Can you work these out from the model? Positions are in its coordinate system, mm. Face numbers are marked on the shaded views. A direction names the side the tool comes from. Round coordinates to 2 decimals unless told otherwise and drop trailing zeros. Order: outer loops, then holes, each group sorted by start corner. A loop starts at its lowest first (then second) coordinate and runs counter-clockwise, first axis right, second up. Notation, with made-up numbers: (36.25, 35) -> (67.25, 35) arc R16 cw to (67.25, 44) -> close; hole circle Ø2 at (-2.5, -31.75). An arc over 180 degrees is marked (long way). One line per item, written item: value.
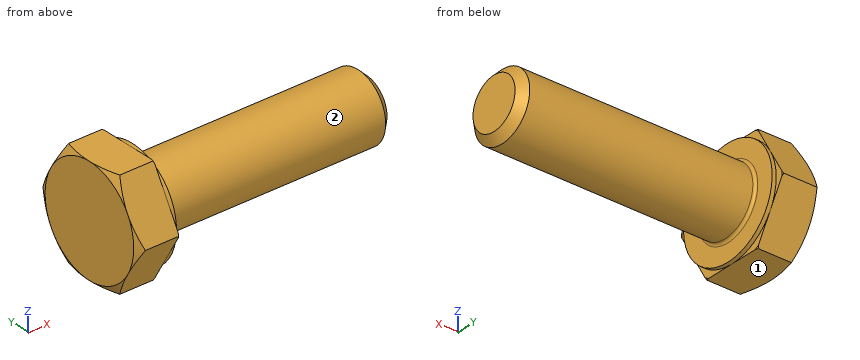
```python
from build123d import *

# Parameters (mm, degrees)
EXTRUDE_368_DEPTH = 6.4
SKETCH_4_W        = 0.6
SKETCH_4_H        = 11.237604307
CHAMFER_1891_SIZE = 1.2
FILLET_1936_R     = 0.4


with BuildPart() as part:
    # 草图1 → Extrude 368 (new body)
    with BuildSketch(Plane(origin=(0, 0, 0), x_dir=(0, 0, -1), z_dir=(1, 0, 0))):
        Polygon((8, 4.618802154), (8, -4.618802154), (0, -9.237604307), (-8, -4.618802154), (-8, 4.618802154), (0, 9.237604307), align=None)
    extrude(amount=EXTRUDE_368_DEPTH)

    # 草图2 → 凸台-旋转1 (revolve)
    with BuildSketch(Plane.XY, mode=Mode.PRIVATE) as revolve_1_sk:
        Polygon((0, 0), (41.4, 0), (41.4, 3.701), (41.4, 5), (0, 5), align=None)
    revolve(revolve_1_sk.sketch.rotate(Axis((0, 0, 0), (1, 0, 0)), 90), axis=Axis((0, 0, 0), (1, 0, 0)))

    # 草图3 → 切除-旋转1 (revolve, cut)
    with BuildSketch(Plane.XY):
        Polygon((0, 8), (3.601282526, 14.237604307), (3.601282526, 19.237604307), (-10, 19.237604307), (-10, 8), align=None)
    revolve(axis=Axis((0, 0, 0), (1, 0, 0)), mode=Mode.SUBTRACT)

    # 草图5 → 切除-旋转2 (revolve, cut)
    with BuildSketch(Plane.XY):
        Polygon((6.4, 8), (2.798717474, 14.237604307), (2.798717474, 19.237604307), (12.798717474, 19.237604307), (12.798717474, 8), align=None)
    revolve(axis=Axis((0, 0, 0), (1, 0, 0)), mode=Mode.SUBTRACT)

    # 草图4 → 切除-旋转3 (revolve, cut)
    with BuildSketch(Plane.XY, mode=Mode.PRIVATE) as cut_revolve_3_sk:
        with Locations((6.1, 13.618802154)):
            Rectangle(SKETCH_4_W, SKETCH_4_H)
    revolve(cut_revolve_3_sk.sketch.rotate(Axis((0, 0, 0), (1, 0, 0)), 270), axis=Axis((0, 0, 0), (1, 0, 0)), mode=Mode.SUBTRACT)

    # Chamfer 1891
    chamfer_1891_edges = [part.edges().sort_by_distance(p)[0] for p in [
        (41.4, 0, -5),
    ]]
    chamfer(chamfer_1891_edges, length=CHAMFER_1891_SIZE)

    # Fillet 1936
    fillet_1936_edges = [part.edges().sort_by_distance(p)[0] for p in [
        (6.4, 0, -5),
    ]]
    fillet(fillet_1936_edges, radius=FILLET_1936_R)


solid = part.part
```
Q1. Please list where these lines run through material, in increasing order: line 1 along X through (y, z) = (6.5, 1); line 2 along Y through (x, z) = (7.5, -3.25); line 3 along Z through (x, y) = (7, 0.25).
Answers below:
line 1: 0 to 6.4
line 2: -3.8 to 3.8
line 3: -4.99 to 4.99
Q2. On a 3-axis mill with a long thin cutter (end or side, diameter ignored), from which of +Z, -Z, +X, -X, +Y, -Y can I reach the whole of each face in a straight line? I mean the marked faces 1 and 2. Say none if no direction works.
Answers below:
face 1: -Z, +X, -X, +Y, -Y
face 2: +X
Q3. I want a section at A-A on x = 35.5. List the corners of the cut face in (y, z) for me.
Answers below:
outline: circle Ø10 at (0, 0)
Q4. Will these pins go through, and if not, where does the flat tip stop? pin 1 Ø1.7 at (y, z) = (8, 0) entering from +X; pin 2 Ø1.5 at (x, z) = (11.5, 4.5) entering from +Y; pin 3 Ø3 at (y, z) = (1, 5) entering from -X; pin 4 Ø0.6 at (y, z) = (-8.5, 0) entering from +X.
Answers below:
pin 1: x = 6.4
pin 2: y = 3.31
pin 3: x = 0
pin 4: x = 5.8
